from build123d import *

# Parameters (mm, degrees)
BRACKET_BODY_DEPTH      = 20
EDGE_FILLETS_R10_R      = 10
MOUNTING_HOLE_SKETCH_R  = 10
MOUNTING_HOLE_CUT_DEPTH = 10


with BuildPart() as part:
    # Bracket Profile Sketch → Bracket Body (new, symmetric)
    with BuildSketch(Plane.XY):
        with BuildLine():
            Line((0, 20), (0, 50))
            Line((0, 50), (30, 50))
            Line((30, 50), (30, 40))
            Line((30, 40), (10, 40))
            Line((10, 40), (10, 20))
            ThreePointArc((10, 20), (12.928932188, 12.928932188), (20, 10))
            Line((20, 10), (50, 10))
            Line((50, 10), (50, 0))
            Line((50, 0), (20, 0))
            ThreePointArc((20, 0), (5.857864376, 5.857864376), (0, 20))
        make_face()
    extrude(amount=BRACKET_BODY_DEPTH, both=True)

    # Edge Fillets R10
    edge_fillets_r10_edges = [part.edges().sort_by_distance(p)[0] for p in [
        (30, 45, -20),
        (30, 45, 20),
    ]]
    fillet(edge_fillets_r10_edges, radius=EDGE_FILLETS_R10_R)

    # Mounting Hole Sketch → Mounting Hole Cut (cut)
    with BuildSketch(Plane.XZ):
        with BuildLine():
            Line((50, 20), (30, 20))
            ThreePointArc((30, 20), (44.142135624, 14.142135624), (50, 0))
            Line((50, 0), (50, 20))
        make_face()
        with BuildLine():
            Line((50, -20), (50, 0))
            ThreePointArc((50, 0), (44.142135624, -14.142135624), (30, -20))
            Line((30, -20), (50, -20))
        make_face()
        with Locations(Location((30, 0, 0), (0, 0, 180))):
            Circle(MOUNTING_HOLE_SKETCH_R)
    extrude(amount=-MOUNTING_HOLE_CUT_DEPTH, mode=Mode.SUBTRACT)


solid = part.part
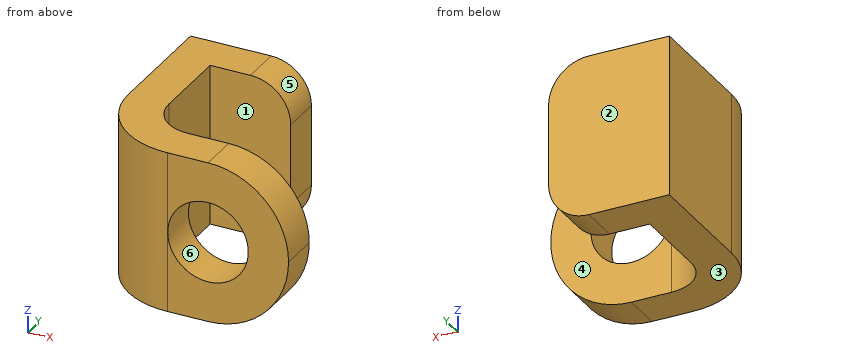
Could you check a few things on this model? Use its own coordinates, in mm. Face numbers are marked on the shaded views. A direction names the side the tool comes from. Coordinates: 2 decimals unless noted, no trailing zeros. Order: outer loops, then holes, each group sorted by start corner. A loop starts at its lowest first (then second) coordinate and runs counter-clockwise, first axis right, second up.
Q1. Suppose I cut it at A-A on x = 18.5. Please give me the cut outline in (y, z).
Q2. Suppose I cut it at C-C on x = 24.5. Please give me the cut outline in (y, z).
Q3. Suppose I cut it at B-B on z = 7. Please give me the cut outline in (x, y) (3 decimals), and give its area (3 significant figures).
Q4. Which directions (+Z, -Z, +X, -X, +Y, -Y) give clear straight access to the entire face, cutting with the end or side of a thin tool? Please do the marked faces 4, 5 and 6.
Q5. Suppose I cut it at D-D on y = 32. Please give me the cut outline in (x, z).
Q6. Will these pins go through, and if not, where does the flat tip stop? pin 1 (8 mm diameter, centred on y = 47.5, z = 3, fed in from +X); pin 2 (5 mm diameter, centred on y = 37, z = -8.5, fed in from +X); pin 3 (2 mm diameter, centred on x = 15, z = -10.5, fed in from -Y).
Q7. Please list where these lines run through material, in increasing order: L1, parallel to Z at x = 30, y = 6; L2, parallel to Y at x = 20.5, z = 13; L3, parallel to Z at x = 24, y = 7.5.
Q8. Thinking about a two-plate mould opening in Y: for the marked faces 1, 2 and 3, which applies, released by +Y, released by -Y, zero draft, split by the parting line, or undercut?
Answer:
1. outline: (0.06, -20) - (10.11, -20) - (10.11, 20) - (0.06, 20) - close; (40, -20) - (50, -20) - (50, 20) - (40, 20) - close
2. outline: (0, -20) - (10, -20) - (10, -8.35) - (0, -8.35) - close; (0, 8.35) - (10, 8.35) - (10, 20) - (0, 20) - close; (40, -18.93) - (50, -18.93) - (50, 18.93) - (40, 18.93) - close
3. outline: (0, 20) arc R20 ccw to (20, 0) - (22.859, 0) - (22.859, 10) - (20, 10) arc R10 cw to (10, 20) - (10, 40) - (30, 40) - (30, 50) - (0, 50) - close; (37.141, 0) - (48.735, 0) - (48.735, 10) - (37.141, 10) - close
3. area: 880 mm2
4. face 4: +Z, -Z, +X
4. face 5: +Z, +X, +Y
4. face 6: -Y
5. outline: (0, -20) - (10, -20) - (10, 20) - (0, 20) - close
6. pin 1: stops at x = 30
6. pin 2: stops at x = 10
6. pin 3: stops at y = 0.4
7. L1: z = -20 to -10, 10 to 20
7. L2: y = 0 to 10, 40 to 50
7. L3: z = -20 to -8, 8 to 20
8. face 1: undercut
8. face 2: released by +Y
8. face 3: zero draft
